from build123d import *

# Parameters (mm, degrees)
BASE_PLATE_SKETCH_W             = 180
BASE_PLATE_SKETCH_H             = 15
BASE_PLATE_DEPTH                = 100
BEARING_UPRIGHT_SKETCH_R        = 30
BEARING_UPRIGHT_SKETCH_R_2      = 15
BEARING_UPRIGHT_DEPTH           = 40
UPRIGHT_BLOCK_SKETCH_W          = 60
UPRIGHT_BLOCK_SKETCH_H          = 51.105876717
UPRIGHT_BLOCK_DEPTH             = 40
BEARING_START                   = -80
BEARING_BORE_SKETCH_R           = 15
BEARING_BORE_DEPTH              = 80
SUPPORT_RIB_A_REACH             = 212.087
SUPPORT_RIB_A_SKETCH_WALL_W     = 492.173009792
SUPPORT_RIB_A_SKETCH_WALL_H     = 10
SUPPORT_RIB_B_REACH             = 212.087
SUPPORT_RIB_B_SKETCH_WALL_W     = 492.173009792
SUPPORT_RIB_B_SKETCH_WALL_H     = 10
BASE_PLATE_CUT_A_SKETCH_R       = 7
BASE_PLATE_CUT_A_DEPTH          = 80
BASE_PLATE_CUT_B_SKETCH_R       = 7
BASE_PLATE_CUT_B_DEPTH          = 222.310106498
BASE_PLATE_CORNER_FILLETS_R10_R = 10


with BuildPart() as part:
    # Base Plate Sketch → Base Plate (new body)
    with BuildSketch(Plane.XY):
        with Locations((90, 7.5)):
            Rectangle(BASE_PLATE_SKETCH_W, BASE_PLATE_SKETCH_H)
    extrude(amount=BASE_PLATE_DEPTH)



with BuildPart() as body_2:
    # Bearing Upright Sketch → Bearing Upright (new, symmetric)
    with BuildSketch(Plane.XY.offset(50)):
        with Locations((90.90588176, 66.105876717)):
            Circle(BEARING_UPRIGHT_SKETCH_R)
        with Locations((90.90588176, 66.105876717)):
            Circle(BEARING_UPRIGHT_SKETCH_R_2, mode=Mode.SUBTRACT)
    extrude(amount=BEARING_UPRIGHT_DEPTH, both=True)


with BuildPart() as part_1:
    add(part.part)

    add(body_2.part)  # Upright Block merges body 2
    # Upright Block Sketch → Upright Block (add, symmetric)
    with BuildSketch(Plane.XY.offset(50)):
        with Locations((90.90588176, 40.552938359)):
            Rectangle(UPRIGHT_BLOCK_SKETCH_W, UPRIGHT_BLOCK_SKETCH_H)
    extrude(amount=UPRIGHT_BLOCK_DEPTH, both=True)

    # Bearing Bore Sketch → Bearing Bore (cut)
    with BuildSketch(Plane.XY.offset(90).offset(BEARING_START)):
        with Locations((90.90588176, 66.105876717)):
            Circle(BEARING_BORE_SKETCH_R)
    extrude(amount=BEARING_BORE_DEPTH, mode=Mode.SUBTRACT)

    # Support Rib A Sketch wall → Support Rib A (add, up to next)
    with BuildSketch(Plane(origin=(37.986107853, 39.654336798, 50), x_dir=(-0.654850683055, -0.755758283383, 0), z_dir=(0.755758283383, -0.654850683055, 0)), mode=Mode.PRIVATE) as support_rib_a_sk1:
        Rectangle(SUPPORT_RIB_A_SKETCH_WALL_W, SUPPORT_RIB_A_SKETCH_WALL_H)
    support_rib_a_tool1 = extrude(support_rib_a_sk1.sketch, amount=SUPPORT_RIB_A_REACH, mode=Mode.PRIVATE) - part_1.part
    add(support_rib_a_tool1.solids().sort_by_distance((37.986107853, 39.654336798, 50))[0])

    # Support Rib B Sketch wall → Support Rib B (add, up to next)
    with BuildSketch(Plane(origin=(145.654619102, 41.357139375, 50), x_dir=(0.707106781187, -0.707106781187, 0), z_dir=(0.707106781187, 0.707106781187, 0)), mode=Mode.PRIVATE) as support_rib_b_sk1:
        Rectangle(SUPPORT_RIB_B_SKETCH_WALL_W, SUPPORT_RIB_B_SKETCH_WALL_H)
    support_rib_b_tool1 = extrude(support_rib_b_sk1.sketch, amount=-SUPPORT_RIB_B_REACH, mode=Mode.PRIVATE) - part_1.part
    add(support_rib_b_tool1.solids().sort_by_distance((145.654619102, 41.357139375, 50))[0])

    # Base Plate Cut A Sketch → Base Plate Cut A (cut)
    with BuildSketch(Plane(origin=(0, 15, 0), x_dir=(1, 0, 0), z_dir=(0, 1, 0))):
        with Locations(Location((20, -20, 0), (0, 0, 270))):
            Circle(BASE_PLATE_CUT_A_SKETCH_R)
    extrude(amount=-BASE_PLATE_CUT_A_DEPTH, mode=Mode.SUBTRACT)

    # Base Plate Cut B Sketch → Base Plate Cut B (cut, through all)
    with BuildSketch(Plane(origin=(0, 15, 0), x_dir=(1, 0, 0), z_dir=(0, 1, 0))):
        with Locations(Location((160, -20, 0), (0, 0, 270))):
            Circle(BASE_PLATE_CUT_B_SKETCH_R)
        with Locations(Location((160, -80, 0), (0, 0, 270))):
            Circle(BASE_PLATE_CUT_B_SKETCH_R)
        with Locations(Location((20, -80, 0), (0, 0, 270))):
            Circle(BASE_PLATE_CUT_B_SKETCH_R)
    extrude(amount=-BASE_PLATE_CUT_B_DEPTH, mode=Mode.SUBTRACT)

    # Base Plate Corner Fillets R10
    base_plate_corner_fillets_r10_edges = [part_1.edges().sort_by_distance(p)[0] for p in [
        (180, 7.5, 100),
        (0, 7.5, 100),
        (180, 7.5, 0),
        (0, 7.5, 0),
    ]]
    fillet(base_plate_corner_fillets_r10_edges, radius=BASE_PLATE_CORNER_FILLETS_R10_R)


solid = part_1.part
Check sheet for the modelled part. Datum: model origin and axes. Units: mm. A direction names the side the tool comes from. Round coordinates to 2 decimals unless told otherwise and drop trailing zeros. Order: outer loops, then holes, each group sorted by start corner. A loop starts at its lowest first (then second) coordinate and runs counter-clockwise, first axis right, second up.
Q1. Scan lines: L1, parallel to X at y = 10, z = 20; L2, parallel to X at y = 6, z = 82; L3, parallel to X at y = 44.5, z = 67. Record each from-to range of solid material in increasing order.
Filled sheet:
L1: x = 0 to 13, 27 to 153, 167 to 180
L2: x = 0 to 13.29, 26.71 to 153.29, 166.71 to 180
L3: x = 60.91 to 120.91
Q2. Draft check along X on faces 4 (the face through (90, 47, 10)), 5 (the face through (79.85, 76.244, 49.44)), 6 (the face through (146.1, 40.91, 49.93)). Enter one of: pulls with the +X half, pulls with the -X half, needs draft (parallel to the pull), parting line crosses it, or undercut.
Filled sheet:
face 4: needs draft
face 5: undercut
face 6: pulls with the +X half
Q3. Cross-section at A-A, the plane z = 20. Enter the section's corners in (x, y).
Filled sheet:
outline: (0, 0) - (13, 0) - (13, 15) - (0, 15) - close; (27, 0) - (153, 0) - (153, 15) - (120.91, 15) - (120.91, 66.11) arc R30 ccw to (60.91, 66.11) - (60.91, 15) - (27, 15) - close; (167, 0) - (180, 0) - (180, 15) - (167, 15) - close; hole circle Ø30 at (90.91, 66.11)
Q4. Cross-section at B-B, the plane z = 65. Enter the section's corners in (x, y), plus the area to 3 significant figures.
Filled sheet:
outline: (0, 0) - (180, 0) - (180, 15) - (120.91, 15) - (120.91, 66.11) arc R30 ccw to (60.91, 66.11) - (60.91, 15) - (0, 15) - close; hole circle Ø30 at (90.91, 66.11)
area: 6,470 mm2
Q5. Cross-section at C-C, the plane x = 160. Enter the section's corners in (y, z), plus the area to 3 significant figures.
Filled sheet:
outline: (0, 0) - (15, 0) - (15, 13) - (0, 13) - close; (0, 27) - (15, 27) - (15, 45) - (27.01, 45) - (27.01, 55) - (15, 55) - (15, 73) - (0, 73) - close; (0, 87) - (15, 87) - (15, 100) - (0, 100) - close
area: 1,200 mm2
Q6. Cross-section at D-D, the plane y = 44. Enter the section's corners in (x, z).
Filled sheet:
outline: (41.75, 45) - (60.91, 45) - (60.91, 10) - (120.91, 10) - (120.91, 45) - (143.01, 45) - (143.01, 55) - (120.91, 55) - (120.91, 90) - (60.91, 90) - (60.91, 55) - (41.75, 55) - close
Q7. Set-up check for faces 1 (the face through (120.906, 40, 28)), 2 (the face through (120.906, 40, 73)), 3 (the face through (46, 35, 55)): record each of +Z, -Z, +X, -X, +Y, -Y from which the full face is reachable in a straight line by a thin tool's end or side.
Filled sheet:
face 1: -Z, +X, +Y
face 2: +Z, +X, +Y
face 3: +Z, -X, +Y
Q8. Depth check by flat-ended pin: P1, Ø4, axis at x = 71, z = 75, coming from the +Y side; P2, Ø12, axis at y = 57, z = 23, coming from the +X side; P3, Ø3, axis at x = 75.5, y = 59.5, coming from the +Z side. Enter the tip coordinate at first touch or a pass-through.
Filled sheet:
P1: stops at y = 90.18
P2: stops at x = 120.91
P3: stops at z = 90
